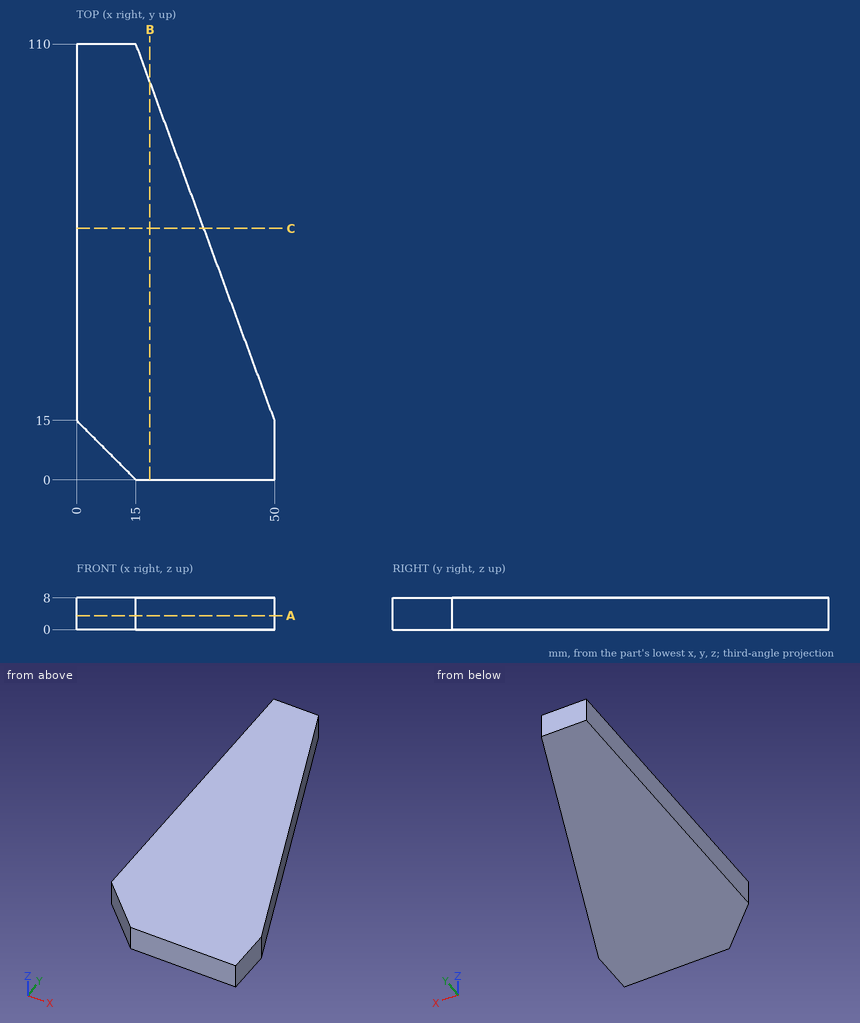
Could you check a few things on this drawing? It's one solid part, dimensions in mm from its lowest x, y, z. Coordinates: 2 decimals unless noted, no trailing zeros. Loops run counter-clockwise (first coordinate to the right, second up) from the corner with the lowest first, then second, coordinate; pieces in that order, holes last.
1. Imagine slicing it at B-B (x = 18.5). Please give me the cut outline in (y, z), and give its area (3 significant figures).
2. I need wall thicknesses on L1, parallel to X at y = 27.5, z = 4.75; L2, parallel to Y at x = 7, z = 4; L3, parallel to X at y = 43, z = 1.5. Which ranges of each line are inside material? Lowest first, please.
3. Imagine slicing it at A-A (z = 3.5). Please give me the cut outline in (x, y), and give its area (4 significant figures).
4. Imagine slicing it at C-C (y = 63.5). Please give me the cut outline in (x, z).
5. For P1, Ø12, axis at x = 29.5, y = 13.5, coming from the -Z side; P2, Ø2, axis at y = 61.5, z = 3, coming from the +X side, each with a flat end and sliding along its axis, tell me the tip position at first contact or that it passes through.
Computed values:
1. outline: (0, 0) - (100.5, 0) - (100.5, 8) - (0, 8) - close
1. area: 804 mm2
2. L1: x = 0 to 45.39
2. L2: y = 8 to 110
2. L3: x = 0 to 39.68
3. outline: (0, 15) - (15, 0) - (50, 0) - (50, 15) - (15, 110) - (0, 110) - close
3. area: 3,725 mm2
4. outline: (0, 0) - (32.13, 0) - (32.13, 8) - (0, 8) - close
5. P1: stops at z = 0
5. P2: stops at x = 33.24
